Here's how the part is built. I have some questions about the finished solid (model axes, mm). A direction names the side the tool comes from. Round coordinates to 2 decimals unless told otherwise and drop trailing zeros. Write each loop counter-clockwise with the first axis right and the second up, starting at its lowest first coordinate (ties: lowest second). Pieces come first, ordered by that corner, then holes. Notation, with made-up numbers: (6.5, -23.75) -> (48.5, -23.75) arc R20 cw to (48.5, -15.75) -> close; hole circle Ø6 at (84.5, 33). An arc over 180 degrees is marked (long way). Answer as CSV lines item,"result".
```python
from build123d import *

# Parameters (mm, degrees)
SKETCH2_W     = 0.2
SKETCH2_H     = 1.6
SKETCH2_W_2   = 0.9
SKETCH2_H_2   = 0.2
CHAMFER1_SIZE = 0.5
CHAMFER2_SIZE = 0.8


with BuildPart() as part:
    # Sketch1 → Revolve1 (revolve)
    with BuildSketch(Plane(origin=(0, 0, 0), x_dir=(1, 0, 0), z_dir=(0, 1, 0))):
        Polygon((0, 0), (0, -4), (10.5, -4), (10.5, -5), (49.5, -5), (49.5, -8), (172.7, -8), (172.7, -4), (196, -4), (196, 0), align=None)
    revolve(axis=Axis((-12.256689328, 0, 0), (1, 0, 0)))

    # Sketch2 → Cut-Revolve1 (revolve, cut)
    with BuildSketch(Plane(origin=(0, 0, 0), x_dir=(1, 0, 0), z_dir=(0, 1, 0))):
        with Locations((52.4, -7.2)):
            Rectangle(SKETCH2_W, SKETCH2_H)
        with Locations((147.6, -7.2)):
            Rectangle(SKETCH2_W, SKETCH2_H)
        with Locations((183.55, -3.9)):
            Rectangle(SKETCH2_W_2, SKETCH2_H_2)
    revolve(axis=Axis((-6.355227553, 0, 0), (1, 0, 0)), mode=Mode.SUBTRACT)

    # Chamfer1
    chamfer1_edges = [part.edges().sort_by_distance(p)[0] for p in [
        (0, 0, -4),
        (196, 0, -4),
        (10.5, 0, -5),
    ]]
    chamfer(chamfer1_edges, length=CHAMFER1_SIZE)

    # Chamfer2
    chamfer2_edges = [part.edges().sort_by_distance(p)[0] for p in [
        (49.5, 0, -8),
    ]]
    chamfer(chamfer2_edges, length=CHAMFER2_SIZE)


solid = part.part
```
1. If I drill on line 1 (X direction, y = -7, z = 1); line 2 (Y direction, x = 162.5, z = 6.25); line 3 (X direction, y = -4, z = -3.5), over which ranges is the centre line in solid material (lowest first)?
Numbers:
line 1,"x = 49.5 to 52.3, 52.5 to 147.5, 147.7 to 172.7"
line 2,"y = -4.99 to 4.99"
line 3,"x = 49.5 to 172.7"
2. For pin 1 Ø5 at (y, z) = (-3, 0) entering from -X; pin 2 Ø2 at (y, z) = (-1.5, 5) entering from -X; pin 3 Ø3 at (x, y) = (43.5, 1) entering from -Z; pin 4 Ø1.5 at (y, z) = (-4.5, -5.5) entering from -X, each with a flat end and sliding along its axis, tell me the tip position at first contact or that it passes through.
Numbers:
pin 1,"stops at x = 0"
pin 2,"stops at x = 10.5"
pin 3,"stops at z = -5"
pin 4,"stops at x = 49.5"
3. On a 3-axis mill with a long thin cutter (end or side, diameter ignored), from which of +Z, -Z, +X, -X, +Y, -Y can I reach the whole of each face in a straight line? I mean faces 1 (the face through (147.7, -7, 0)), 2 (the face through (0, 0, 0)), 3 (the face through (30.52, 4.88, -1.08)), 4 (the face through (189.83, 3.905, -0.867)). Say none if no direction works.
Numbers:
face 1,"none"
face 2,"+Z, -Z, -X, +Y, -Y"
face 3,"-X"
face 4,"+X"
4. If we mould it in two halves opening along X, with no side actions, what happens to faces 5 (the face through (183.556, -0.167, -3.796)), 6 (the face through (10.5, 3, 3)), 7 (the face through (51.31, 7.81, -1.73)), 8 (the face through (172.7, 2, -4))? For each: released by +X, released by -X, zero draft, split by the parting line, or undercut.
Numbers:
face 5,"undercut"
face 6,"released by -X"
face 7,"zero draft"
face 8,"released by +X"
5. Suppose I cut it at A-A on x = 95. Please give me the cut outline in (y, z), and give its area (3 significant figures).
Numbers:
outline,"circle Ø16 at (0, 0)"
area,"201 mm^2"
